The listing builds one solid part. Answer for the finished solid, in the listing's coordinates (mm). A direction names the side the tool comes from. Coordinates: 2 decimals unless noted, no trailing zeros. Order: outer loops, then holes, each group sorted by start corner. A loop starts at its lowest first (then second) coordinate and runs counter-clockwise, first axis right, second up. Notation, with made-up numbers: (18, 76) -> (37, 76) arc R34 ccw to (37, 111) -> close; hole circle Ø9 at (59, 73). An arc over 180 degrees is marked (long way). Write item = value, one per line.
from build123d import *

# Parameters (mm, degrees)
EXTRUDE1_DEPTH     = 8
SKETCH3_OUTSIDE_W  = 150.432
SKETCH3_OUTSIDE_H  = 150.432
SKETCH3_OUTSIDE_R  = 9.5
CUT_EXTRUDE1_DEPTH = 10
CUT_EXTRUDE1_DRAFT = -80
FILLET1_R          = 1


with BuildPart() as part:
    # Sketch1 → Revolve1 (revolve)
    with BuildSketch(Plane.XY, mode=Mode.PRIVATE) as revolve1_sk:
        Polygon((16, 10.4775), (16, 9.3155), (12, 9.3155), (12, 13), (8, 13), (8, 1.5), (0, 1.5), (0, 0), (26, 0), (26, 9.3155), (24.838, 10.4775), align=None)
    revolve(revolve1_sk.sketch.rotate(Axis((0, 0, 0), (1, 0, 0)), 90), axis=Axis((0, 0, 0), (1, 0, 0)))

    # Sketch2 → Extrude1 (add)
    with BuildSketch(Plane.ZY):
        Polygon((0, 10.969655115), (-9.5, 5.484827557), (-9.5, -5.484827557), (0, -10.969655115), (9.5, -5.484827557), (9.5, 5.484827557), align=None)
    extrude(amount=-EXTRUDE1_DEPTH)


with BuildPart() as cut_extrude1_tool:
    # Sketch3 outside → Cut-Extrude1 (with draft: the straight prism first)
    with BuildSketch(Plane.ZY):
        Rectangle(SKETCH3_OUTSIDE_W, SKETCH3_OUTSIDE_H)
        Circle(SKETCH3_OUTSIDE_R, mode=Mode.SUBTRACT)
    extrude(amount=-CUT_EXTRUDE1_DEPTH)
    # Cut-Extrude1: the draft: its side faces are tilted about the plane it starts from
    cut_extrude1_sides = [cut_extrude1_tool.faces().sort_by_distance(p)[0] for p in [
        (5, -75.216, 0),
        (5, 0, 75.216),
        (5, 75.216, 0),
        (5, 0, -75.216),
        (5, 0, -9.5),
    ]]
    draft(cut_extrude1_sides, Plane.ZY, CUT_EXTRUDE1_DRAFT)


with BuildPart() as part_1:
    add(part.part)

    # Cut-Extrude1: cut by cut_extrude1_tool
    add(cut_extrude1_tool.part, mode=Mode.SUBTRACT)

    # Fillet1
    fillet1_edges = [part_1.edges().sort_by_distance(p)[0] for p in [
        (16, 0, -9.3155),
        (12, 0, -9.3155),
    ]]
    fillet(fillet1_edges, radius=FILLET1_R)


solid = part_1.part
Q1. The mould has two halves that part along X. Classify faces 1 (the face through (4, 0, -9.5)), 2 (the face through (26, 0, 0)), 3 (the face through (13.986, -2.798, 8.885)), 4 (the face through (0.06, -9.85, -0.02)): released by +X, released by -X, zero draft, split by the parting line, or undercut.
The answers:
face_1 = zero draft
face_2 = released by +X
face_3 = undercut
face_4 = released by -X
Q2. A tool of negligible diameter and unlimited length cuts with its end or side. For faces 5 (the face through (3.9, 8.2, 4.8)), 6 (the face through (20.36, -10.39, -1.36)), 7 (the face through (3.9, -8.2, -4.8)), 8 (the face through (4, 0, 9.5)), 9 (the face through (3.944, 8.266, -4.684)), from which of +Z, -Z, +X, -X, +Y, -Y can it reach the whole face along a straight path? Write none if from no direction.
The answers:
face_5 = +Z, -X, +Y
face_6 = +X
face_7 = -Z, -X, -Y
face_8 = +Z, -X, +Y, -Y
face_9 = -Z, -X, +Y
Q3. Section A-A, the plane x = 1.5 is taken. Give the vertices of the cut face in (y, z).
The answers:
outline = (-10.97, 0) -> (-5.48, -9.5) -> (5.48, -9.5) -> (10.97, 0) -> (5.48, 9.5) -> (-5.48, 9.5) -> close
Q4. Each of these flat-tipped pins is pushed along its axis until it touches: pin 1 Ø5 at (x, y) = (18.5, 8.5) entering from +Z; pin 2 Ø1 at (x, z) = (20.5, 3.5) entering from +Y; pin 3 Ø3 at (x, z) = (21.5, 2) entering from -Y. Where does it stop, or does it pass through?
The answers:
pin_1 = 8.59
pin_2 = 10.04
pin_3 = -10.47
Q5. Section C-C, the plane z = 11.25 is taken. Give the vertices of the cut face in (x, y).
The answers:
outline = (8, -6.51) -> (12, -6.51) -> (12, 6.51) -> (8, 6.51) -> close
Q6. Find the intervals of material crossed by line 1 along X through (y, z) = (3, -10.5); line 2 along X through (y, z) = (-5.5, 8.5); line 3 along X through (y, z) = (-3.5, -9.25), in increasing order.
The answers:
line_1 = 8 to 12
line_2 = 0.11 to 12.02, 15.98 to 25.19
line_3 = 0.07 to 12.1, 15.9 to 25.43
Q7. Section D-D, the plane x = 18.75 is taken. Give the vertices of the cut face in (y, z) (1 decimal), plus the area to 3 significant figures.
The answers:
outline = circle Ø21 at (0, 0)
area = 345 mm2
Q8. Section B-B, the plane x = 13.75 is taken. Give the vertices of the cut face in (y, z).
The answers:
outline = circle Ø18.63 at (0, 0)
